Can you work these out from the model? Positions are in its coordinate system, mm. A direction names the side the tool comes from. Give positions to 0.01 mm unless a question says otherwise; leave off trailing zeros. Order: outer loops, then holes, each group sorted by start corner. A loop starts at its lowest first (then second) coordinate and runs counter-clockwise, first axis right, second up. Notation, with made-up numbers: M 79,12 L 138,12 A36 cw 138,51 Z; hole C 83,-31.75 d6. An arc over 180 degrees is marked long. Answer as a JSON object with one key per item and string values.
```python
from build123d import *

# Parameters (mm, degrees)
BOSS_EXTRUDE1_DEPTH = 800
CUT_EXTRUDE1_DEPTH  = 800
CUT_EXTRUDE2_DEPTH  = 803.081458262


with BuildPart() as part:
    # Sketch1 → Boss-Extrude1 (new body)
    with BuildSketch(Plane.XY):
        with BuildLine():
            Line((-25.764376508, 0), (-25.764376508, -15))
            Line((-25.764376508, -15), (-55.764376508, -15))
            Line((-55.764376508, -15), (-55.764376508, 0))
            ThreePointArc((-55.764376508, 0), (-40.764376508, 15), (-25.764376508, 0))
        make_face()
    extrude(amount=BOSS_EXTRUDE1_DEPTH)

    # Sketch2 → Cut-Extrude1 (cut)
    with BuildSketch(Plane.XY.offset(800)):
        with BuildLine():
            Line((-27.264376508, 0), (-27.264376508, -9))
            Line((-27.264376508, -9), (-54.264376508, -9))
            Line((-54.264376508, -9), (-54.264376508, 0))
            ThreePointArc((-54.264376508, 0), (-40.764376508, 13.5), (-27.264376508, 0))
        make_face()
    extrude(amount=-CUT_EXTRUDE1_DEPTH, mode=Mode.SUBTRACT)

    # Sketch3 → Cut-Extrude2 (cut, through all)
    with BuildSketch(Plane.XY.offset(800)):
        Polygon((-51.764376508, -15), (-51.764376508, -13.5), (-53.264376508, -13.5), (-53.264376508, -10.5), (-28.264376508, -10.5), (-28.264376508, -13.5), (-29.764376508, -13.5), (-29.764376508, -15), align=None)
    extrude(amount=-CUT_EXTRUDE2_DEPTH, mode=Mode.SUBTRACT)


solid = part.part
```
1) For faces 1 (the face through (-41, -9, 406)), 2 (the face through (-41, -10, 0)), which set-ups out of +Z, -Z, +X, -X, +Y, -Y let a thin tool reach every point of the face, with its end or its side?
Results found:
{"face 1": "+Z, -Z", "face 2": "-Z, +X, -X, +Y, -Y"}
2) I'm going to push flat-ended pins straight in: pin 1 Ø5 at (y, z) = (3.5, 590) entering from -X; pin 2 Ø1.2 at (x, z) = (-28.5, 405) entering from +Y; pin 3 Ø10 at (x, z) = (-50.5, 640.5) entering from +Y. Where does each tip first touch, or does it pass through?
Results found:
{"pin 1": "stops at x = -55.73", "pin 2": "stops at y = 9.43", "pin 3": "stops at y = 14.23"}
3) I want a section at B-B on x = -35.25. Write out the boundary of the cut face in (y, z), and give its area (3 significant figures).
Results found:
{"outline": "M -10.5,0 L -9,0 L -9,800 L -10.5,800 Z; M 12.32,0 L 13.95,0 L 13.95,800 L 12.32,800 Z", "area": "2,500 mm²"}
4) I need wall thicknesses on L1, parallel to X at y = -13, z = 460; L2, parallel to X at y = -3, z = 381; L3, parallel to Y at x = -52.5, z = 760.5. Which ranges of each line are inside material? Lowest first, please.
Results found:
{"L1": "x = -55.76 to -53.26, -28.26 to -25.76", "L2": "x = -55.76 to -54.26, -27.26 to -25.76", "L3": "y = -15 to -13.5, -10.5 to -9, 6.67 to 9.34"}
5) I want a section at A-A on z = 120. Write out the boundary of the cut face in (x, y), and give its area (3 significant figures).
Results found:
{"outline": "M -55.76,-15 L -51.76,-15 L -51.76,-13.5 L -53.26,-13.5 L -53.26,-10.5 L -28.26,-10.5 L -28.26,-13.5 L -29.76,-13.5 L -29.76,-15 L -25.76,-15 L -25.76,0 A15 ccw -55.76,0 Z; hole M -54.26,-9 L -27.26,-9 L -27.26,0 A13.5 ccw -54.26,0 Z", "area": "166 mm²"}
